```python
from build123d import *

# Parameters (mm, degrees)
SKETCH1_W           = 88.5
SKETCH1_H           = 46
SKETCH1_R           = 1.6
BOSS_EXTRUDE1_DEPTH = 2
CUT_EXTRUDE1_DEPTH  = 50.910544978
FILLET1_R           = 2


with BuildPart() as part:
    # Sketch1 → Boss-Extrude1 (new body)
    with BuildSketch(Plane(origin=(0, 0, 0), x_dir=(1, 0, 0), z_dir=(0, 1, 0))):
        Rectangle(SKETCH1_W, SKETCH1_H)
        with Locations(Location((-41.25, -5.5, 0), (0, 0, 270))):
            Circle(SKETCH1_R, mode=Mode.SUBTRACT)
        with Locations(Location((-41.25, -15.5, 0), (0, 0, 270))):
            Circle(SKETCH1_R, mode=Mode.SUBTRACT)
        with Locations(Location((41.25, -15.5, 0), (0, 0, 90))):
            Circle(SKETCH1_R, mode=Mode.SUBTRACT)
        with Locations(Location((41.25, -5.5, 0), (0, 0, 90))):
            Circle(SKETCH1_R, mode=Mode.SUBTRACT)
        with Locations(Location((-8.75, -20, 0), (0, 0, 270))):
            Circle(SKETCH1_R, mode=Mode.SUBTRACT)
        with Locations(Location((1.25, -20, 0), (0, 0, 270))):
            Circle(SKETCH1_R, mode=Mode.SUBTRACT)
        with Locations(Location((-34, 17, 0), (0, 0, 270))):
            Circle(SKETCH1_R, mode=Mode.SUBTRACT)
        with Locations(Location((-21, 17, 0), (0, 0, 270))):
            Circle(SKETCH1_R, mode=Mode.SUBTRACT)
        with Locations(Location((21, 17, 0), (0, 0, 270))):
            Circle(SKETCH1_R, mode=Mode.SUBTRACT)
        with Locations(Location((34, 17, 0), (0, 0, 270))):
            Circle(SKETCH1_R, mode=Mode.SUBTRACT)
        with Locations(Location((1.25, 20, 0), (0, 0, 90))):
            Circle(SKETCH1_R, mode=Mode.SUBTRACT)
        with Locations(Location((-8.75, 20, 0), (0, 0, 90))):
            Circle(SKETCH1_R, mode=Mode.SUBTRACT)
    extrude(amount=BOSS_EXTRUDE1_DEPTH)

    # Sketch2 → Cut-Extrude1 (cut, through all)
    with BuildSketch(Plane(origin=(0, 2, 0), x_dir=(1, 0, 0), z_dir=(0, 1, 0))):
        with BuildLine():
            Line((-27.75, 10), (-27.75, -13))
            ThreePointArc((-27.75, -13), (-31.25, -16.5), (-34.75, -13))
            Line((-34.75, -13), (-34.75, 10))
            ThreePointArc((-34.75, 10), (-31.25, 13.5), (-27.75, 10))
        make_face()
        with BuildLine():
            Line((-15.25, 10), (-15.25, -13))
            ThreePointArc((-15.25, -13), (-18.75, -16.5), (-22.25, -13))
            Line((-22.25, -13), (-22.25, 10))
            ThreePointArc((-22.25, 10), (-18.75, 13.5), (-15.25, 10))
        make_face()
        with BuildLine():
            Line((-2.75, 13), (-2.75, -13))
            ThreePointArc((-2.75, -13), (-6.25, -16.5), (-9.75, -13))
            Line((-9.75, -13), (-9.75, 13))
            ThreePointArc((-9.75, 13), (-6.25, 16.5), (-2.75, 13))
        make_face()
        with BuildLine():
            Line((9.75, 13), (9.75, -13))
            ThreePointArc((9.75, -13), (6.25, -16.5), (2.75, -13))
            Line((2.75, -13), (2.75, 13))
            ThreePointArc((2.75, 13), (6.25, 16.5), (9.75, 13))
        make_face()
        with BuildLine():
            Line((22.25, 10), (22.25, -13))
            ThreePointArc((22.25, -13), (18.75, -16.5), (15.25, -13))
            Line((15.25, -13), (15.25, 10))
            ThreePointArc((15.25, 10), (18.75, 13.5), (22.25, 10))
        make_face()
        with BuildLine():
            Line((34.75, 10), (34.75, -13))
            ThreePointArc((34.75, -13), (31.25, -16.5), (27.75, -13))
            Line((27.75, -13), (27.75, 10))
            ThreePointArc((27.75, 10), (31.25, 13.5), (34.75, 10))
        make_face()
    extrude(amount=-CUT_EXTRUDE1_DEPTH, mode=Mode.SUBTRACT)

    # Fillet1
    fillet1_edges = [part.edges().sort_by_distance(p)[0] for p in [
        (44.25, 1, 23),
        (-44.25, 1, 23),
        (-44.25, 1, -23),
        (44.25, 1, -23),
    ]]
    fillet(fillet1_edges, radius=FILLET1_R)


solid = part.part
```
Build history of the part. All positions in model axes, mm. A direction names the side the tool comes from. Give positions to 0.01 mm unless a question says otherwise; leave off trailing zeros. Order: outer loops, then holes, each group sorted by start corner. A loop starts at its lowest first (then second) coordinate and runs counter-clockwise, first axis right, second up. Notation, with made-up numbers: M 45,-39.5 L 76,-39.5 A22 ccw 76,-29.5 Z; hole C -3.5,63 d3. An arc over 180 degrees is marked long. Return JSON: item names as keys, results as strings.
Q1. 3-axis set-ups, long thin cutter, end or side, ignore diameter. For faces 5 (the face through (9.75, 1, 0)), 6 (the face through (-43.68, 1.01, 22.4)): which of +Z, -Z, +X, -X, +Y, -Y reach the whole face in a straight line?
Answer list:
{"face 5": "+Y, -Y", "face 6": "+Z, -X, +Y, -Y"}
Q2. Flat gauge pin, fed straight in: pin 1 (3 mm diameter, centred on x = 41.25, z = 15.5, fed in from -Y). Where does the tip first touch, or does it go through?
Answer list:
{"pin 1": "passes through"}
Q3. Band-saw the part on C-C (x = 41.25). Give the cut face in (y, z), then the cut area to 3 significant figures.
Answer list:
{"outline": "M 0,-23 L 2,-23 L 2,3.9 L 0,3.9 Z; M 0,7.1 L 2,7.1 L 2,13.9 L 0,13.9 Z; M 0,17.1 L 2,17.1 L 2,23 L 0,23 Z", "area": "79.2 mm^2"}
Q4. Band-saw the part on B-B (z = 9). Give the cut face in (x, y).
Answer list:
{"outline": "M -44.25,0 L -34.75,0 L -34.75,2 L -44.25,2 Z; M -27.75,0 L -22.25,0 L -22.25,2 L -27.75,2 Z; M -15.25,0 L -9.75,0 L -9.75,2 L -15.25,2 Z; M -2.75,0 L 2.75,0 L 2.75,2 L -2.75,2 Z; M 9.75,0 L 15.25,0 L 15.25,2 L 9.75,2 Z; M 22.25,0 L 27.75,0 L 27.75,2 L 22.25,2 Z; M 34.75,0 L 44.25,0 L 44.25,2 L 34.75,2 Z"}
Q5. Band-saw the part on D-D (y = 1.05). Count the separate pieces of the cut face and the enclosed holes in it, then the cut area to 3 significant figures.
Answer list:
{"separate pieces": "1", "enclosed holes": "18", "area": "2,730 mm^2"}
Q6. Two-plate mould, pull along X, no slides. Class faces 1 (the face through (-1, 1, 23)), 2 (the face through (-34.75, 1, 2)), 3 (the face through (44.25, 1, 0)), 4 (the face through (-44.25, 1, 0)): pulls with the +X half, pulls with the -X half, needs draft (parallel to the pull), parting line crosses it, or undercut.
Answer list:
{"face 1": "needs draft", "face 2": "undercut", "face 3": "pulls with the +X half", "face 4": "pulls with the -X half"}
Q7. Band-saw the part on A-A (x = 6.25). Give the cut face in (y, z).
Answer list:
{"outline": "M 0,-23 L 2,-23 L 2,-16.5 L 0,-16.5 Z; M 0,16.5 L 2,16.5 L 2,23 L 0,23 Z"}
Q8. Wall check: probe 1 along Z at (x, y) = (41.25, 1.2); probe 2 along X at (y, z) = (1.45, -20); probe 3 along X at (y, z) = (1.45, -17). Give the ranges that are in metal, low to high. Write a range as from..to.
Answer list:
{"probe 1": "z = -23..3.9, 7.1..13.9, 17.1..23", "probe 2": "x = -44.25..-10.35, -7.15..-0.35, 2.85..44.25", "probe 3": "x = -44.25..-35.6, -32.4..-22.6, -19.4..19.4, 22.6..32.4, 35.6..44.25"}
